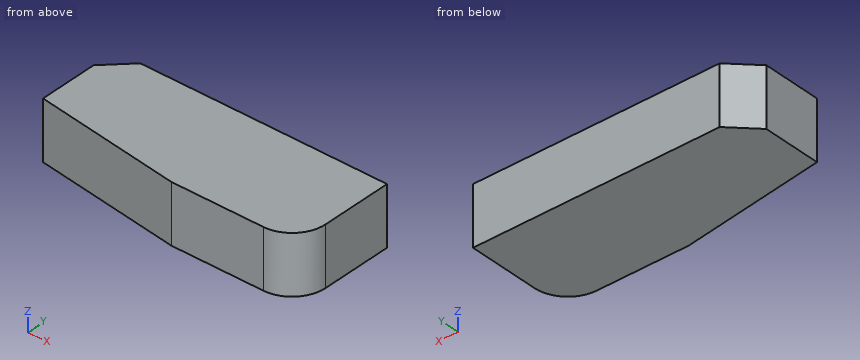
```python
from build123d import *

# Parameters (mm, degrees)
EXTRUDE_1_DEPTH = 7
CHAMFER_1_SIZE  = 6
FILLET_1_R      = 8


with BuildPart() as part:
    # 草图1 → 凸台-拉伸1 (new, symmetric)
    with BuildSketch(Plane.XY):
        Polygon((0, 5), (0, 25), (65, 25), (65, 0), (35, 0), align=None)
    extrude(amount=EXTRUDE_1_DEPTH, both=True)

    # 倒角1
    chamfer_1_edges = [part.edges().sort_by_distance(p)[0] for p in [
        (0, 25, 0),
    ]]
    chamfer(chamfer_1_edges, length=CHAMFER_1_SIZE)

    # 圆角1
    fillet_1_edges = [part.edges().sort_by_distance(p)[0] for p in [
        (65, 0, 0),
    ]]
    fillet(fillet_1_edges, radius=FILLET_1_R)


solid = part.part
```
Part model, mm, in its own coordinate system. Give positions to 0.01 mm unless a question says otherwise; leave off trailing zeros. Write each loop counter-clockwise with the first axis right and the second up, starting at its lowest first coordinate (ties: lowest second). Pieces come first, ordered by that corner, then holes. Notation, with made-up numbers: (-31.5, 13) -> (7.5, 13) arc R17 ccw to (7.5, 23) -> close; hole circle Ø10 at (13.25, 84.5). An arc over 180 degrees is marked (long way). Put each result on its own line as item: value. Start each with the question number.
Item 1: Wall check: L1, parallel to Y at x = 59, z = -0.5; L2, parallel to X at y = 23.5, z = 4.5; L3, parallel to X at y = 7.5, z = -1.75. Give the ranges that are in metal, low to high. Write a range as [from, to].
Item 2: Cut at A-A (z = 5.5). List the corners of the cut face in (x, y).
Item 3: Pin check, flat tips, straight feed: pin 1 Ø1 at (y, z) = (6.5, -4) entering from +X; pin 2 Ø4 at (y, z) = (4, -4) entering from +X; pin 3 Ø5 at (x, z) = (31.5, -5) entering from -Y. Stop position of each tip, or through.
Item 4: Cut at C-C (x = 22). List the corners of the cut face in (y, z), then the cut area to 3 significant figures.
Item 5: Cut at B-B (y = 21.75). List the corners of the cut face in (x, z), then the cut area to 4 significant figures.
Answer list:
1. L1: y = [0.25, 25]
1. L2: x = [4.5, 65]
1. L3: x = [0, 64.98]
2. outline: (0, 5) -> (35, 0) -> (57, 0) arc R8 ccw to (65, 8) -> (65, 25) -> (6, 25) -> (0, 19) -> close
3. pin 1: stops at x = 64.94
3. pin 2: stops at x = 64.75
3. pin 3: stops at y = 0.14
4. outline: (1.86, -7) -> (25, -7) -> (25, 7) -> (1.86, 7) -> close
4. area: 324 mm2
5. outline: (2.75, -7) -> (65, -7) -> (65, 7) -> (2.75, 7) -> close
5. area: 871.5 mm2
